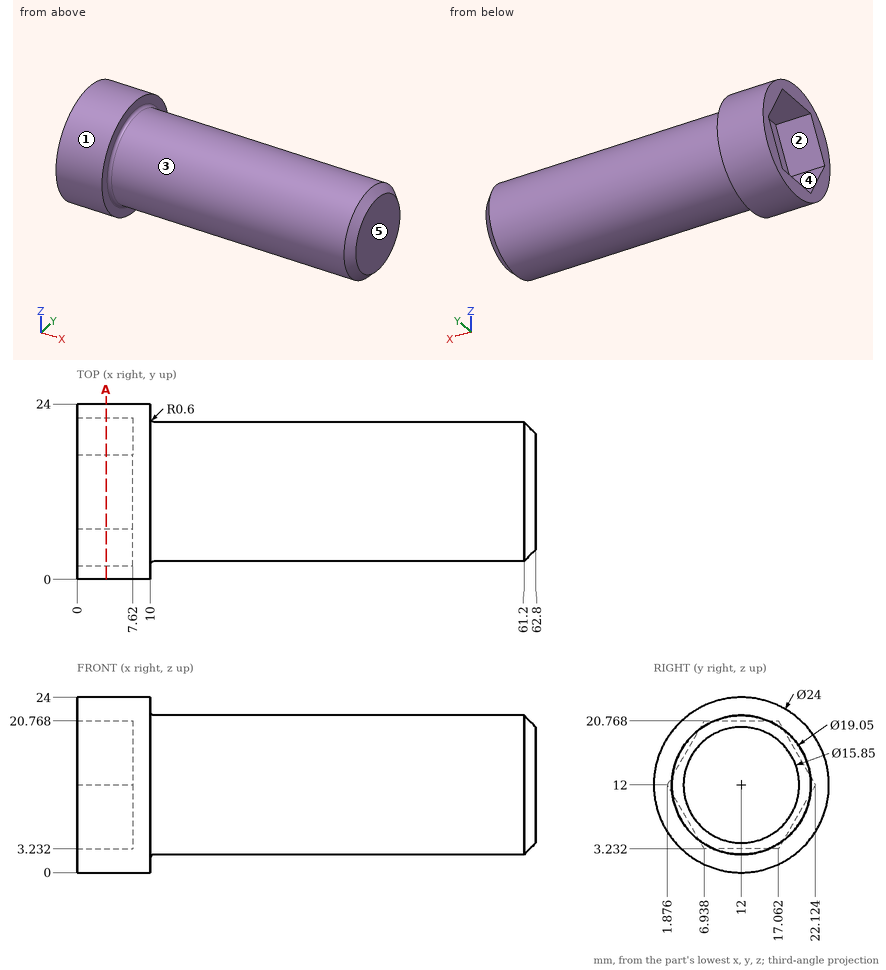
Check sheet for the drawn part. Datum: minimum x, y, z corner. Units: mm. A direction names the side the tool comes from. Coordinates: 2 decimals unless noted, no trailing zeros. Order: outer loops, then holes, each group sorted by start corner. A loop starts at its lowest first (then second) coordinate and runs counter-clockwise, first axis right, second up. Notation, with made-up numbers: (30.5, 49) -> (35.5, 49) arc R8 cw to (35.5, 58) -> close; hole circle Ø2 at (41.25, 86.25). An arc over 180 degrees is marked (long way). Use a Markdown table: item, result. Add a question column.
1. Go/stop test with flat-tipped pins: pin 1 Ø5 at (y, z) = (6.5, 14) entering from -X; pin 2 Ø8 at (x, z) = (12, 8) entering from +Y; pin 3 Ø1 at (x, z) = (28.5, 6) entering from -Y; pin 4 Ø10 at (y, z) = (11, 6.5) entering from -X. Record where each tip stops, or that it passes through.
2. Mould release check, pull along Y, two halves, no side actions. Record for the marked faces 3, 4 and 5: pulls with the +Y half, pulls with the -Y half, needs draft (parallel to the pull), parting line crosses it, or undercut.
3. Material ranges on L1, parallel to X at y = 18.25, z = 13; L2, parallel to X at y = 7, z = 2.25; L3, parallel to Y at x = 6.5, z = 6.25 (1 decimal), recorded low to high.
4. Set-up check for the marked faces 1 and 2: record each of +Z, -Z, +X, -X, +Y, -Y from which the full face is reachable in a straight line by a thin tool's end or side.
5. Cross-section at A-A (x = 4). Enter the section's corners in (y, z).
Filled sheet:
| question | item | result |
|---|---|---|
| 1 | pin 1 | x = 7.62 |
| 1 | pin 2 | y = 23.99 |
| 1 | pin 3 | y = 4.22 |
| 1 | pin 4 | x = 0 |
| 2 | face 3 | parting line crosses it |
| 2 | face 4 | undercut |
| 2 | face 5 | needs draft |
| 3 | L1 | 7.62 to 62.8 |
| 3 | L2 | 0 to 10 |
| 3 | L3 | 1.5 to 5.2, 18.8 to 22.5 |
| 4 | face 1 | +X, -X |
| 4 | face 2 | -X |
| 5 | outline | circle Ø24 at (12, 12); hole (1.88, 12) -> (6.94, 3.23) -> (17.06, 3.23) -> (22.12, 12) -> (17.06, 20.77) -> (6.94, 20.77) -> close |
